Can you work these out from the model? Positions are in its coordinate system, mm. Coordinates: 2 decimals unless noted, no trailing zeros. Order: outer loops, then holes, each group sorted by start corner. A loop starts at its lowest first (then second) coordinate and runs counter-clockwise, first axis right, second up. Notation, with made-up numbers: (35.25, 83.5) - (49.25, 83.5) arc R29 cw to (49.25, 107.5) - close; hole circle Ø3 at (-15, 55.5). An arc over 180 degrees is marked (long way). Use a Markdown table: item, result. Add a question column.
(1) I want a section at D-D (x = -45.5). List the corners of the cut face in (y, z) for me.
(2) If I drill on L1, parallel to Y at x = 0, z = 5.25; L2, parallel to Y at x = 43, z = 1; L3, parallel to Y at x = -3, z = 0.5, over which ranges is the centre line in solid material (lowest first)? Write a range as [from, to].
(3) I want a section at A-A (y = 6.5). List the corners of the cut face in (x, z) for me.
(4) For pin 1 Ø1.5 at (y, z) = (-9.5, 6.5) entering from -X; pin 2 Ø1.5 at (x, z) = (64.5, 5) entering from -Y; pin 3 Ø4 at (x, z) = (-20.5, 5.5) entering from -Y, each with a flat end and sliding along its axis, tell me the tip position at first contact or that it passes through.
(5) I want a section at C-C (z = 4.25). List the corners of the cut face in (x, y) for me, and give its area (3 significant figures).
(6) I want a section at B-B (x = 0). List the corners of the cut face in (y, z) for me, and give its area (3 significant figures).
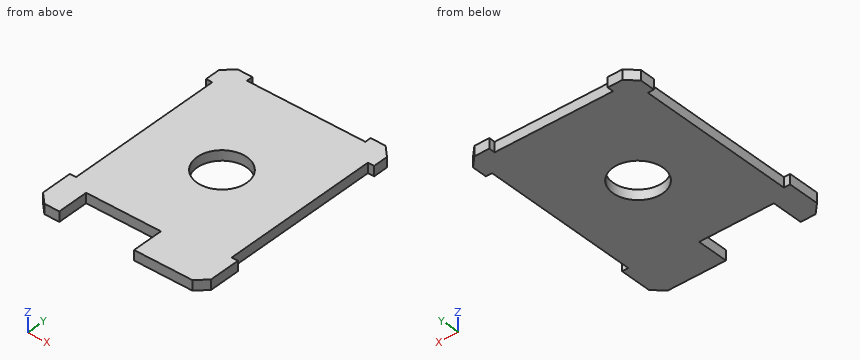
```python
from build123d import *

# Parameters (mm, degrees)
SKETCH_1_W          = 135
SKETCH_1_H          = 180
EXTRUDE_1_DEPTH     = 8
CUT_EXTRUDE_1_REACH = 114.784
SKETCH_2_W          = 95
SKETCH_2_H          = 5
SKETCH_2_W_2        = 60
SKETCH_2_H_2        = 25
SKETCH_2_W_3        = 5
SKETCH_2_H_3        = 127
CHAMFER_1_SIZE      = 8
CUT_EXTRUDE_2_REACH = 114.784
SKETCH_3_R          = 20


with BuildPart() as part:
    # 草图1 → 凸台-拉伸1 (new body)
    with BuildSketch(Plane.XY):
        Rectangle(SKETCH_1_W, SKETCH_1_H)
    extrude(amount=EXTRUDE_1_DEPTH)

    # 草图2 → 切除-拉伸1 (cut, up to next)
    with BuildSketch(Plane.XY.offset(8), mode=Mode.PRIVATE) as cut_extrude_1_sk1:
        with Locations((0, 87.5)):
            Rectangle(SKETCH_2_W, SKETCH_2_H)
    cut_extrude_1_tool1 = extrude(cut_extrude_1_sk1.sketch, amount=-CUT_EXTRUDE_1_REACH, mode=Mode.PRIVATE) & part.part
    # 草图2 → 切除-拉伸1 (cut, up to next)
    with BuildSketch(Plane.XY.offset(8), mode=Mode.PRIVATE) as cut_extrude_1_sk2:
        with Locations((-17.5, -77.5)):
            Rectangle(SKETCH_2_W_2, SKETCH_2_H_2)
    cut_extrude_1_tool2 = extrude(cut_extrude_1_sk2.sketch, amount=-CUT_EXTRUDE_1_REACH, mode=Mode.PRIVATE) & part.part
    # 草图2 → 切除-拉伸1 (cut, up to next)
    with BuildSketch(Plane.XY.offset(8), mode=Mode.PRIVATE) as cut_extrude_1_sk3:
        with Locations((-65, 6.5)):
            Rectangle(SKETCH_2_W_3, SKETCH_2_H_3)
    cut_extrude_1_tool3 = extrude(cut_extrude_1_sk3.sketch, amount=-CUT_EXTRUDE_1_REACH, mode=Mode.PRIVATE) & part.part
    # 草图2 → 切除-拉伸1 (cut, up to next)
    with BuildSketch(Plane.XY.offset(8), mode=Mode.PRIVATE) as cut_extrude_1_sk4:
        with Locations((65, 6.5)):
            Rectangle(SKETCH_2_W_3, SKETCH_2_H_3)
    cut_extrude_1_tool4 = extrude(cut_extrude_1_sk4.sketch, amount=-CUT_EXTRUDE_1_REACH, mode=Mode.PRIVATE) & part.part
    add(cut_extrude_1_tool1.solids().sort_by_distance((0, 87.5, 8))[0], mode=Mode.SUBTRACT)
    add(cut_extrude_1_tool2.solids().sort_by_distance((-17.5, -77.5, 8))[0], mode=Mode.SUBTRACT)
    add(cut_extrude_1_tool3.solids().sort_by_distance((-65, 6.5, 8))[0], mode=Mode.SUBTRACT)
    add(cut_extrude_1_tool4.solids().sort_by_distance((65, 6.5, 8))[0], mode=Mode.SUBTRACT)

    # 倒角1
    chamfer_1_edges = [part.edges().sort_by_distance(p)[0] for p in [
        (67.5, -90, 4),
        (-67.5, -90, 4),
        (-67.5, 90, 4),
        (67.5, 90, 4),
    ]]
    chamfer(chamfer_1_edges, length=CHAMFER_1_SIZE)

    # 草图3 → 切除-拉伸2 (cut, up to next)
    with BuildSketch(Plane.XY.offset(8), mode=Mode.PRIVATE) as cut_extrude_2_sk1:
        with Locations((0, 6.5)):
            Circle(SKETCH_3_R)
    cut_extrude_2_tool1 = extrude(cut_extrude_2_sk1.sketch, amount=-CUT_EXTRUDE_2_REACH, mode=Mode.PRIVATE) & part.part
    add(cut_extrude_2_tool1.solids().sort_by_distance((0, 6.5, 8))[0], mode=Mode.SUBTRACT)


solid = part.part
```
Answers follow:
| question | item | result |
|---|---|---|
| 1 | outline | (-65, 0) - (85, 0) - (85, 8) - (-65, 8) - close |
| 2 | L1 | y = [-65, -13.5], [26.5, 85] |
| 2 | L2 | y = [-90, 85] |
| 2 | L3 | y = [-65, -13.27], [26.27, 85] |
| 3 | outline | (-62.5, 0) - (-20, 0) - (-20, 8) - (-62.5, 8) - close; (20, 0) - (62.5, 0) - (62.5, 8) - (20, 8) - close |
| 4 | pin 1 | stops at x = -62.5 |
| 4 | pin 2 | stops at y = -85.75 |
| 4 | pin 3 | stops at y = -65 |
| 5 | outline | (-67.5, -82) - (-59.5, -90) - (-47.5, -90) - (-47.5, -65) - (12.5, -65) - (12.5, -90) - (59.5, -90) - (67.5, -82) - (67.5, -57) - (62.5, -57) - (62.5, 70) - (67.5, 70) - (67.5, 82) - (59.5, 90) - (47.5, 90) - (47.5, 85) - (-47.5, 85) - (-47.5, 90) - (-59.5, 90) - (-67.5, 82) - (-67.5, 70) - (-62.5, 70) - (-62.5, -57) - (-67.5, -57) - close; hole circle Ø40 at (0, 6.5) |
| 5 | area | 19,700 mm² |
| 6 | outline | (-65, 0) - (-13.5, 0) - (-13.5, 8) - (-65, 8) - close; (26.5, 0) - (85, 0) - (85, 8) - (26.5, 8) - close |
| 6 | area | 880 mm² |
